Part model, mm, in its own coordinate system. Face numbers are marked on the shaded views. A direction names the side the tool comes from. Give positions to 0.01 mm unless a question says otherwise; leave off trailing zeros. Write each loop counter-clockwise with the first axis right and the second up, starting at its lowest first coordinate (ties: lowest second). Pieces come first, ordered by that corner, then holes. Notation, with made-up numbers: M 57,-36.75 L 73,-36.75 A27 cw 73,0.25 Z; hole C 16.5,36.5 d5. An arc over 180 degrees is marked long. Use CSV: the item, a comma, the result in double quotes. Start each with the question number.
1. Band-saw the part on A-A, the plane x = -11.5. List the corners of the cut face in (y, z), then the cut area to 3 significant figures.
2. Drop flat-ended pins along their axis: pin 1 Ø4 at (x, z) = (-0.5, -9) entering from +Y; pin 2 Ø1.5 at (x, z) = (6, -2) entering from -Y; pin 3 Ø4.5 at (x, z) = (11.5, 14.5) entering from -Y; pin 4 Ø1.5 at (y, z) = (3, -7.5) entering from +X. Give the stop position or say it passes through.
3. Band-saw the part on C-C, the plane y = 5.2. List the corners of the cut face in (x, z).
4. Drill centre lines: line 1 along X through (y, z) = (1.85, 14.5); line 2 along X through (y, z) = (0.4, -8); line 3 along X through (y, z) = (4.35, -8). Where is each one in solid material? Low to high. Write a range as from..to.
5. Mould opens along X. For the marked faces 4, 5 and 6 say: pulls with the +X half, pulls with the -X half, needs draft (parallel to the pull), parting line crosses it, or undercut.
6. Band-saw the part on B-B, the plane x = 11.5. List the corners of the cut face in (y, z).
7. Band-saw the part on D-D, the plane z = -14. List the corners of the cut face in (x, y).
8. 3-axis set-ups, long thin cutter, end or side, ignore diameter. For the marked faces 1, 2 and 3: which of +Z, -Z, +X, -X, +Y, -Y reach the whole face in a straight line?
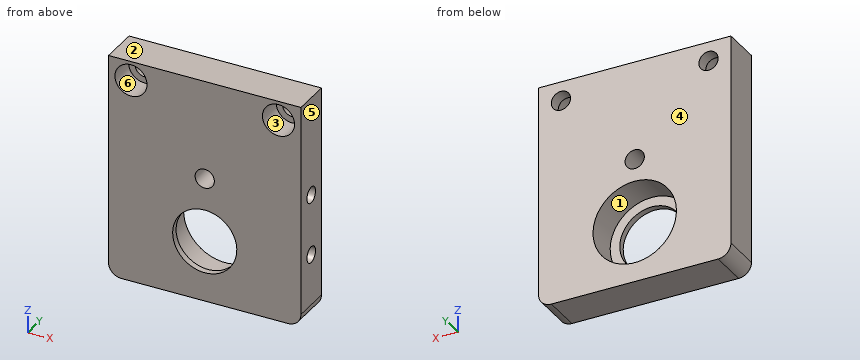
from build123d import *

# Parameters (mm, degrees)
SKETCH1_R             = 5
SKETCH1_R_2           = 1.5
BOSS_EXTRUDE1_DEPTH   = 6
SKETCH3_R             = 6.5
CUT_EXTRUDE1_DEPTH    = 5
SKETCH4_R             = 1.5
CUT_EXTRUDE2_DEPTH    = 24.817010728
SKETCH5_R             = 2.5
CUT_EXTRUDE3_DEPTH    = 4
SKETCH8_R             = 1
CUT_EXTRUDE6_DEPTH    = 2
M3_TAPPED_HOLE1_D     = 2.5
M3_TAPPED_HOLE1_DEPTH = 7.5
M3_TAPPED_HOLE1_TIP   = 0.751075774


with BuildPart() as part:
    # Sketch1 → Boss-Extrude1 (new body)
    with BuildSketch(Plane(origin=(0, 0, 0), x_dir=(1, 0, 0), z_dir=(0, 1, 0))):
        with BuildLine():
            Line((-13, 17.5), (13, 17.5))
            ThreePointArc((13, 17.5), (14.414213562, 16.914213562), (15, 15.5))
            Line((15, 15.5), (15, -17.5))
            Line((15, -17.5), (-15, -17.5))
            Line((-15, -17.5), (-15, 15.5))
            ThreePointArc((-15, 15.5), (-14.414213562, 16.914213562), (-13, 17.5))
        make_face()
        with Locations(Location((0, 8, 0), (0, 0, 270))):
            Circle(SKETCH1_R, mode=Mode.SUBTRACT)
        with Locations(Location((0, -2, 0), (0, 0, 270))):
            Circle(SKETCH1_R_2, mode=Mode.SUBTRACT)
    extrude(amount=BOSS_EXTRUDE1_DEPTH)

    # Sketch3 → Cut-Extrude1 (cut)
    with BuildSketch(Plane(origin=(0, 6, 0), x_dir=(1, 0, 0), z_dir=(0, 1, 0))):
        with Locations(Location((0, 8, 0), (0, 0, 270))):
            Circle(SKETCH3_R)
    extrude(amount=-CUT_EXTRUDE1_DEPTH, mode=Mode.SUBTRACT)

    # Sketch4 → Cut-Extrude2 (cut, through all)
    with BuildSketch(Plane(origin=(0, 6, 0), x_dir=(1, 0, 0), z_dir=(0, 1, 0))):
        with Locations(Location((-11.5, -14.5, 0), (0, 0, 270))):
            Circle(SKETCH4_R)
        with Locations(Location((11.5, -14.5, 0), (0, 0, 270))):
            Circle(SKETCH4_R)
    extrude(amount=-CUT_EXTRUDE2_DEPTH, mode=Mode.SUBTRACT)

    # Sketch5 → Cut-Extrude3 (cut)
    with BuildSketch(Plane.XZ):
        with Locations(Location((11.5, 14.5, 0), (0, 0, 270))):
            Circle(SKETCH5_R)
        with Locations(Location((-11.5, 14.5, 0), (0, 0, 270))):
            Circle(SKETCH5_R)
    extrude(amount=-CUT_EXTRUDE3_DEPTH, mode=Mode.SUBTRACT)

    # Sketch8 → Cut-Extrude6 (cut)
    with BuildSketch(Plane(origin=(15, 0, 0), x_dir=(0, 0, -1), z_dir=(1, 0, 0))):
        with Locations((-2, 3)):
            Circle(SKETCH8_R)
        with Locations((7.5, 3)):
            Circle(SKETCH8_R)
    extrude(amount=-CUT_EXTRUDE6_DEPTH, mode=Mode.SUBTRACT)

    # M3 Tapped Hole1
    with Locations(Plane(origin=(15, 0, 0), x_dir=(0, 0, -1), z_dir=(1, 0, 0))):
        with Locations((-2, 3), (7.5, 3)):
            Hole(M3_TAPPED_HOLE1_D / 2, depth=M3_TAPPED_HOLE1_DEPTH)
            with Locations((0, 0, -(M3_TAPPED_HOLE1_DEPTH + M3_TAPPED_HOLE1_TIP / 2))):  # 118° drill point
                Cone(0, M3_TAPPED_HOLE1_D / 2, M3_TAPPED_HOLE1_TIP, mode=Mode.SUBTRACT)


solid = part.part
Output:
1,outline,"M 0,-17.5 L 6,-17.5 L 6,13 L 4,13 L 4,12 L 0,12 Z; M 0,17 L 4,17 L 4,16 L 6,16 L 6,17.5 L 0,17.5 Z"
1,area,"184 mm²"
2,pin 1,"passes through"
2,pin 2,"stops at y = 0"
2,pin 3,"stops at y = 4"
2,pin 4,"stops at x = 7.2"
3,outline,"M -15,-15.5 A2 ccw -13,-17.5 L 13,-17.5 A2 ccw 15,-15.5 L 15,17.5 L -15,17.5 Z; hole C -11.5,14.5 d3; hole C 0,-8 d13; hole C 0,2 d3; hole C 11.5,14.5 d3"
4,line 1,"x = -15..-14, -9..9, 14..15"
4,line 2,"x = -15..-5, 5..15"
4,line 3,"x = -15..-6.5, 6.5..15"
5,face 4,"needs draft"
5,face 5,"pulls with the +X half"
5,face 6,"undercut"
6,outline,"M 0,-17.5 L 6,-17.5 L 6,13 L 4,13 L 4,12 L 0,12 Z; M 0,17 L 4,17 L 4,16 L 6,16 L 6,17.5 L 0,17.5 Z; hole C 3,-7.5 d2.5; hole C 3,2 d2.5"
7,outline,"M -15,0 L 15,0 L 15,6 L 2.5,6 L 2.5,1 L -2.5,1 L -2.5,6 L -15,6 Z"
8,face 1,"+Y"
8,face 2,"+Z, +X, -X, +Y, -Y"
8,face 3,"-Y"
